```python
from build123d import *

# Parameters (mm, degrees)
SKETCH1_R           = 10
BOSS_EXTRUDE1_DEPTH = 240
SKETCH2_W           = 30
SKETCH2_H           = 30
BOSS_EXTRUDE2_DEPTH = 5
SKETCH3_R           = 4.5
CUT_EXTRUDE1_DEPTH  = 38
FILLET1_R           = 5
FILLET2_R           = 5
SKETCH4_R           = 4
CUT_EXTRUDE2_DEPTH  = 20


with BuildPart() as part:
    # Sketch1 → Boss-Extrude1 (new body)
    with BuildSketch(Plane.XY):
        Circle(SKETCH1_R)
    extrude(amount=BOSS_EXTRUDE1_DEPTH)

    # Sketch2 → Boss-Extrude2 (add, symmetric)
    with BuildSketch(Plane(origin=(0, 0, 0), x_dir=(0, 0, -1), z_dir=(1, 0, 0))):
        with Locations((15, 0)):
            Rectangle(SKETCH2_W, SKETCH2_H)
    extrude(amount=BOSS_EXTRUDE2_DEPTH, both=True)

    # Sketch3 → Cut-Extrude1 (cut)
    with BuildSketch(Plane(origin=(5, 0, 0), x_dir=(0, 0, -1), z_dir=(1, 0, 0))):
        with Locations((15, 0)):
            Circle(SKETCH3_R)
    extrude(amount=-CUT_EXTRUDE1_DEPTH, mode=Mode.SUBTRACT)

    # Fillet1
    fillet1_edges = [part.edges().sort_by_distance(p)[0] for p in [
        (0, -15, -30),
        (0, 15, -30),
    ]]
    fillet(fillet1_edges, radius=FILLET1_R)

    # Fillet2
    fillet2_edges = [part.edges().sort_by_distance(p)[0] for p in [
        (-10, 0, 240),
    ]]
    fillet(fillet2_edges, radius=FILLET2_R)

    # Sketch4 → Cut-Extrude2 (cut)
    with BuildSketch(Plane.XY.offset(240)):
        Circle(SKETCH4_R)
    extrude(amount=-CUT_EXTRUDE2_DEPTH, mode=Mode.SUBTRACT)


solid = part.part
```
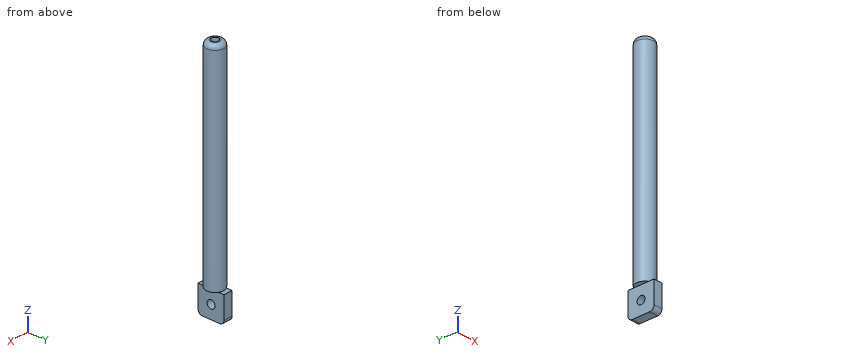
Source: CAD feature listing. Evaluate the final solid. Frame: model axes, mm. Give positions to 0.01 mm unless a question says otherwise; leave off trailing zeros. Order: outer loops, then holes, each group sorted by start corner. A loop starts at its lowest first (then second) coordinate and runs counter-clockwise, first axis right, second up.
(1) Material intervals for line 1 along Y through (x, z) = (0, 233.5); line 2 along Z through (x, y) = (0, 0.5); line 3 along Y through (x, z) = (-0.25, -15), sorted ascending.
(2) Section query B-B (z = 223). Return the cut outline in (x, y), plus the area to 3 significant figures.
(3) Section query A-A (z = -15). Return the cut outline in (x, y), plus the area to 3 significant figures.
(4) Section query C-C (z = 118.5). Return the cut outline in (x, y).
(5) Section query D-D (y = -12.75). Return the cut outline in (x, z).
(6) Contact query for flat-ended pins moving along their axis: P1, Ø1, axis at x = 1, y = -9.5, coming from the +Z side; P2, Ø1.9, axis at x = -1.5, y = 11, coming from the +Z side; P3, Ø4, axis at x = 6.5, z = 171, coming from the +Y side; P4, Ø8, axis at y = 0, z = -15, coming from the +X side. Output: stop coordinate, or through.
Outcome:
1. line 1: y = -10 to -4, 4 to 10
1. line 2: z = -30 to -19.47, -10.53 to 220
1. line 3: y = -15 to -4.5, 4.5 to 15
2. outline: circle Ø20 at (0, 0); hole circle Ø8 at (0, 0)
2. area: 264 mm2
3. outline: (-5, -15) - (5, -15) - (5, -4.5) - (-5, -4.5) - close; (-5, 4.5) - (5, 4.5) - (5, 15) - (-5, 15) - close
3. area: 210 mm2
4. outline: circle Ø20 at (0, 0)
5. outline: (-5, -29.18) - (5, -29.18) - (5, 0) - (-5, 0) - close
6. P1: stops at z = 237.93
6. P2: stops at z = 0
6. P3: stops at y = 8.93
6. P4: passes through
